Model file for the job. Use its own axes, mm. Face numbers are marked on the shaded views. A direction names the side the tool comes from. Give positions to 0.01 mm unless a question says otherwise; leave off trailing zeros. Order: outer loops, then holes, each group sorted by start corner. A loop starts at its lowest first (then second) coordinate and runs counter-clockwise, first axis right, second up. Notation, with made-up numbers: (24, 58) -> (67, 58) arc R16 cw to (67, 66) -> close; hole circle Ø1 at (20.25, 19). An arc over 180 degrees is marked (long way). Use CSV: the item, a comma, the result in double quotes. Start each with the question number.
1. Cut at A-A on y = 0. List the corners of the cut face in (x, z).
2. Drop flat-ended pins along their axis: pin 1 (5 mm diameter, centred on x = -1.5, z = 2.5, fed in from +Y); pin 2 (1 mm diameter, centred on x = -2, z = 9, fed in from +Y); pin 3 (1 mm diameter, centred on x = -5, z = 7.5, fed in from +Y) (1 decimal); pin 4 (5 mm diameter, centred on y = -4.5, z = 20.5, fed in from +X). Give the stop position or say it passes through.
3. 3-axis set-ups, long thin cutter, end or side, ignore diameter. For the marked faces 1 and 2: which of +Z, -Z, +X, -X, +Y, -Y reach the whole face in a straight line?
4. Wall check: line 1 (Z direction, x = 4.5, y = -0.75); line 2 (Y direction, x = 0.25, z = 18); line 3 (Y direction, x = 2.5, z = 20.5). Give the ranges that are in metal, low to high. Write a range as from..to.
5. Cut at C-C on z = 18.75. List the corners of the cut face in (x, y).
6. Pull direction Z, two halves, no side cores. Call the marked faces 3, 4 and 5: released by +Z, released by -Z, zero draft, split by the parting line, or undercut.
7. Cut at D-D on z = 7.75. List the corners of the cut face in (x, y).
```python
from build123d import *

# Parameters (mm, degrees)
SKETCH1_R           = 4.5
BOSS_EXTRUDE1_DEPTH = 1
SKETCH2_R           = 4
BOSS_EXTRUDE2_DEPTH = 1
SKETCH3_R           = 4
BOSS_EXTRUDE3_DEPTH = 14
SKETCH4_R           = 5
BOSS_EXTRUDE4_DEPTH = 3
SKETCH5_R           = 6.5
BOSS_EXTRUDE5_DEPTH = 6
CHAMFER1_SIZE       = 0.5


with BuildPart() as part:
    # Sketch1 → Boss-Extrude1 (new body)
    with BuildSketch(Plane.XY):
        Circle(SKETCH1_R)
    extrude(amount=BOSS_EXTRUDE1_DEPTH)

    # Sketch2 → Boss-Extrude2 (add)
    with BuildSketch(Plane.XY.offset(1)):
        Circle(SKETCH2_R)
    extrude(amount=BOSS_EXTRUDE2_DEPTH)

    # Sketch3 → Boss-Extrude3 (add)
    with BuildSketch(Plane.XY.offset(2)):
        Circle(SKETCH3_R)
    extrude(amount=BOSS_EXTRUDE3_DEPTH)

    # Sketch4 → Boss-Extrude4 (add)
    with BuildSketch(Plane.XY.offset(16)):
        Circle(SKETCH4_R)
    extrude(amount=BOSS_EXTRUDE4_DEPTH)

    # Sketch5 → Boss-Extrude5 (add)
    with BuildSketch(Plane.XY.offset(19)):
        Circle(SKETCH5_R)
    extrude(amount=BOSS_EXTRUDE5_DEPTH)

    # Chamfer1
    chamfer1_edges = [part.edges().sort_by_distance(p)[0] for p in [
        (-6.5, 0, 19),
        (-6.5, 0, 25),
        (-4.5, 0, 0),
    ]]
    chamfer(chamfer1_edges, length=CHAMFER1_SIZE)


solid = part.part
```
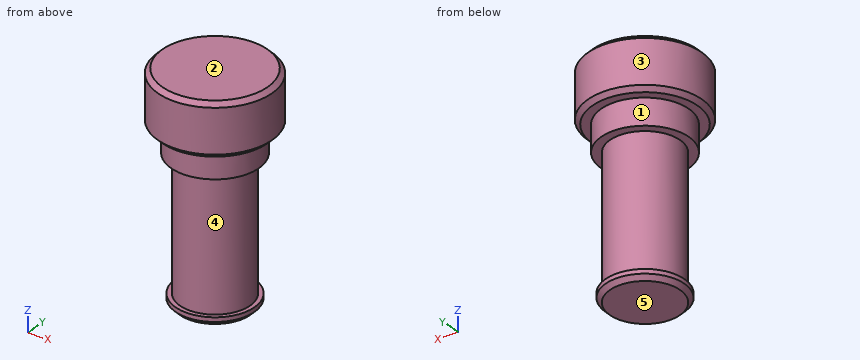
Verdict:
1,outline,"(-6.5, 19.5) -> (-6, 19) -> (-5, 19) -> (-5, 16) -> (-4, 16) -> (-4, 1) -> (-4.5, 1) -> (-4.5, 0.5) -> (-4, 0) -> (4, 0) -> (4.5, 0.5) -> (4.5, 1) -> (4, 1) -> (4, 16) -> (5, 16) -> (5, 19) -> (6, 19) -> (6.5, 19.5) -> (6.5, 24.5) -> (6, 25) -> (-6, 25) -> (-6.5, 24.5) -> close"
2,pin 1,"y = 4.5"
2,pin 2,"y = 3.71"
2,pin 3,"through"
2,pin 4,"x = 6.18"
3,face 1,"-Z"
3,face 2,"+Z, +X, -X, +Y, -Y"
4,line 1,"16..25"
4,line 2,"-4.99..4.99"
4,line 3,"-6..6"
5,outline,"circle Ø10 at (0, 0)"
6,face 3,"zero draft"
6,face 4,"undercut"
6,face 5,"released by -Z"
7,outline,"circle Ø8 at (0, 0)"
